Geometry check sheet. Reference: the model listing, model coordinates, mm. A direction names the side the tool comes from. Round coordinates to 2 decimals unless told otherwise and drop trailing zeros. Order: outer loops, then holes, each group sorted by start corner. A loop starts at its lowest first (then second) coordinate and runs counter-clockwise, first axis right, second up. Notation, with made-up numbers: (-26.5, -13) - (27.5, -13) arc R17 cw to (27.5, 1) - close; hole circle Ø9 at (65.25, 49.5). An arc over 180 degrees is marked (long way). Return JSON: item names as keys, results as strings. Group by question number.
Q1. Gauge pin test, flat ends, axial feed: pin 1 Ø16 at (x, z) = (21.5, 132) entering from +Y; pin 2 Ø21.5 at (y, z) = (22, 66) entering from -X; pin 3 Ø8.5 at (x, y) = (28.5, 23.5) entering from +Z; pin 4 Ø5 at (x, y) = (-28.5, 21) entering from -Z. Record the tip position at first contact, or that the pin passes through.
Q2. Draft check along Z on faces 1 (the cylindrical face through (0.532, 54.138, 41.056)), 2 (the flat face through (26, -5, 79)), 3 (the flat face through (0.08, 41.8, 104.44)), 4 (the flat face through (-1, 17, 0)). Enter one of: pulls with the +Z half, pulls with the -Z half, needs draft (parallel to the pull), parting line crosses it, or undercut.
Q3. Material ranges on line 1 along Y through (x, z) = (1, 30); line 2 along X through (y, z) = (24.5, 7); line 3 along Y through (x, z) = (8.5, 25), recorded low to high.
Q4. Tool access check on faces 5 (the flat face through (-38, 23, 43)), 6 (the flat face through (22, 30, 60)), 7 (the flat face through (-22, 15.829, 111)), 8 (the flat face through (38, 21, 43)). Record the directions out of +Z, -Z, +X, -X, +Y, -Y that give a thin tool (end or side, any length) a straight path to the whole face; none if there is none.
Q5. Sectioned sample at B-B, the plane x = 28.5. Record the cut outline in (y, z).
Q6. Sectioned sample at A-A, the plane y = -3.5. Record the cut outline in (x, z), then the cut area to 3 significant figures.
Q7. Sectioned sample at C-C, the plane x = -12. Record the cut outline in (y, z).
Q8. Sectioned sample at D-D, the plane z = 92. Record the cut outline in (x, y), then the cut area to 3 significant figures.
```python
from build123d import *

# Parameters (mm, degrees)
BASE_SLIDE_PROFILE_SKETCH_W     = 76
BASE_SLIDE_PROFILE_SKETCH_H     = 60
BASE_BLOCK_160_DEPTH            = 160
BEARING_BLOCK_SHAPING_CUT_DEPTH = 198.027916804
SUPPORT_RIB_12_DEPTH            = 6
BORE_SKETCH_R                   = 15
BORE_30_DEPTH                   = 198.027916804


with BuildPart() as part:
    # Base Slide Profile Sketch → Base Block 160 (new body)
    with BuildSketch(Plane.XY):
        Polygon((-26, -10), (-26, 0), (26, 0), (26, -10), (50, -10), (50, 2), (38, 2), (38, 14), (-38, 14), (-38, 2), (-50, 2), (-50, -10), align=None)
        with Locations((0, 44)):
            Rectangle(BASE_SLIDE_PROFILE_SKETCH_W, BASE_SLIDE_PROFILE_SKETCH_H)
    extrude(amount=BASE_BLOCK_160_DEPTH)

    # Bearing Block Outline Sketch → Bearing Block Shaping Cut (cut, through all)
    with BuildSketch(Plane(origin=(38, 0, 0), x_dir=(0, 0, -1), z_dir=(1, 0, 0))):
        with BuildLine():
            Line((-60, 15.828860139), (-60, 44))
            ThreePointArc((-60, 44), (-51.213203403, 65.213203468), (-29.999999908, 74))
            Line((-29.999999908, 74), (-160, 74))
            Line((-160, 74), (-160, 15.828860139))
            Line((-160, 15.828860139), (-60, 15.828860139))
        make_face()
        with BuildLine():
            Line((0, 74), (-29.999999908, 74))
            ThreePointArc((-29.999999908, 74), (-8.786796532, 65.213203403), (0, 44))
            Line((0, 44), (0, 74))
        make_face()
    extrude(amount=-BEARING_BLOCK_SHAPING_CUT_DEPTH, mode=Mode.SUBTRACT)

    # Support Rib Sketch → Support Rib 12 (add, symmetric)
    with BuildSketch(Plane(origin=(0, 0, 0), x_dir=(0, 0, -1), z_dir=(1, 0, 0))):
        with BuildLine():
            Line((-160, 15.828860139), (-47.311623158, 68.501177597))
            ThreePointArc((-47.311623158, 68.501177597), (-56.639713725, 57.795856357), (-60, 44))
            Line((-60, 44), (-60, 15.828860139))
            Line((-60, 15.828860139), (-160, 15.828860139))
        make_face()
    extrude(amount=SUPPORT_RIB_12_DEPTH, both=True)

    # Bore Sketch → Bore Ø30 (cut, through all)
    with BuildSketch(Plane(origin=(38, 0, 0), x_dir=(0, 0, -1), z_dir=(1, 0, 0))):
        with Locations((-30, 44)):
            Circle(BORE_SKETCH_R)
    extrude(amount=-BORE_30_DEPTH, mode=Mode.SUBTRACT)


solid = part.part
```
Reply:
{
 "1": {"pin 1": "y = 15.83", "pin 2": "x = -38", "pin 3": "z = 60", "pin 4": "z = 0"},
 "2": {"face 1": "undercut", "face 2": "needs draft", "face 3": "pulls with the +Z half", "face 4": "pulls with the -Z half"},
 "3": {"line 1": "0 to 29, 59 to 74", "line 2": "-38 to 38", "line 3": "0 to 29.86, 58.14 to 73.58"},
 "4": {"face 5": "+Z, -Z, -X, +Y", "face 6": "+Z, +X, +Y", "face 7": "+Z, -X, +Y", "face 8": "+Z, -Z, +X, +Y"},
 "5": {"outline": "(-10, 0) - (44, 0) arc R30 ccw to (44, 60) - (15.83, 60) - (15.83, 160) - (-10, 160) - close; hole circle Ø30 at (44, 30)"},
 "6": {"outline": "(-50, 0) - (-26, 0) - (-26, 160) - (-50, 160) - close; (26, 0) - (50, 0) - (50, 160) - (26, 160) - close", "area": "7,680 mm^2"},
 "7": {"outline": "(0, 0) - (44, 0) arc R30 ccw to (44, 60) - (15.83, 60) - (15.83, 160) - (0, 160) - close; hole circle Ø30 at (44, 30)"},
 "8": {"outline": "(-50, -10) - (-26, -10) - (-26, 0) - (26, 0) - (26, -10) - (50, -10) - (50, 2) - (38, 2) - (38, 15.83) - (6, 15.83) - (6, 47.61) - (-6, 47.61) - (-6, 15.83) - (-38, 15.83) - (-38, 2) - (-50, 2) - close", "area": "2,110 mm^2"}
}
